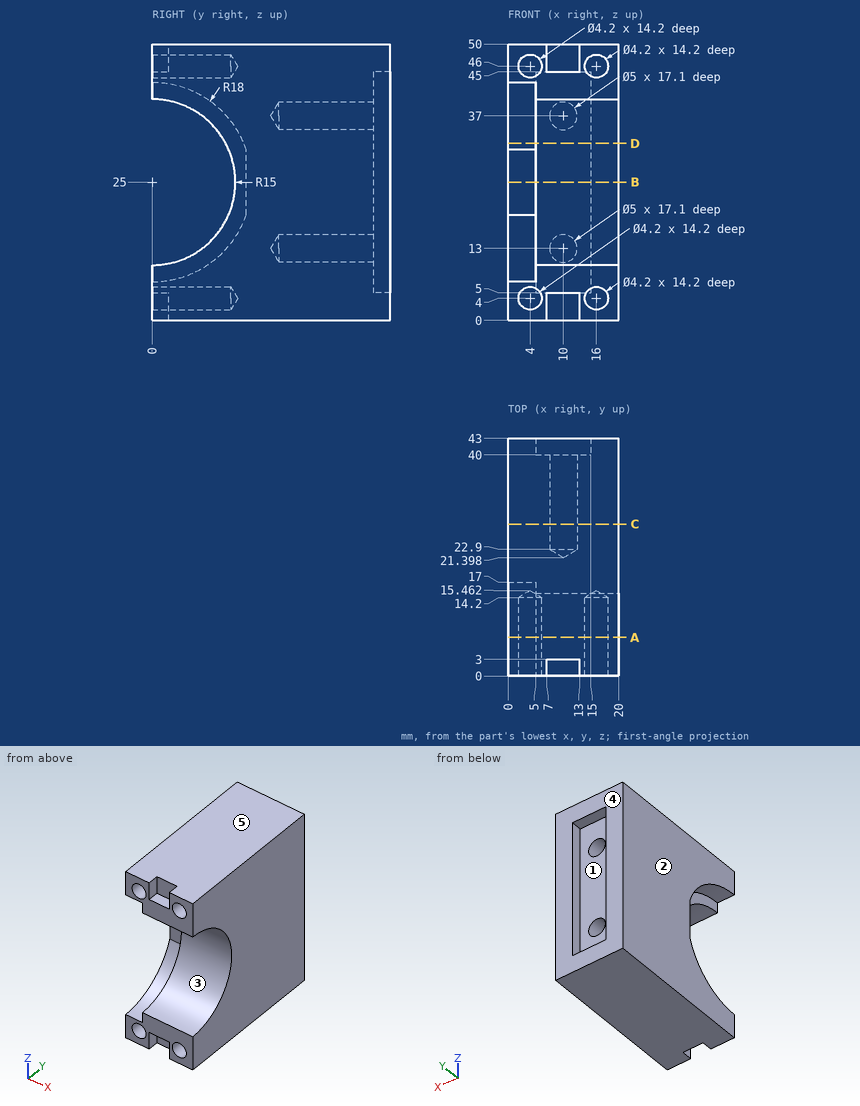
Study the drawing (mm; zero at the part's minimum x, y, z) and answer. A direction names the side the tool comes from. Coordinates: 2 decimals unless noted, no trailing zeros. Loops run counter-clockwise (first coordinate to the right, second up) from the corner with the lowest first, then second, coordinate; pieces in that order, holes last. Notation, with made-up numbers: (-22.5, -14.5) -> (26.5, -14.5) arc R32 ccw to (26.5, 14.5) -> close; hole circle Ø10 at (78, -14.75). An arc over 180 degrees is marked (long way). Answer as CSV lines item,"result".
1) For a pull along Z with two mould halves and no side action, classify the marked faces 3, 4 and 5 as released by +Z, released by -Z, zero draft, split by the parting line, or undercut.
A:
face 3,"undercut"
face 4,"zero draft"
face 5,"released by +Z"
2) The part is cut by section B-B (z = 25). Give the vertices of the cut face in (x, y), and give its area (3 significant figures).
A:
outline,"(0, 17) -> (5, 17) -> (5, 15) -> (20, 15) -> (20, 43) -> (15, 43) -> (15, 40) -> (5, 40) -> (5, 43) -> (0, 43) -> close"
area,"520 mm²"
3) The part is cut by section D-D (z = 32). Give the vertices of the cut face in (x, y).
A:
outline,"(0, 16.58) -> (5, 16.58) -> (5, 13.27) -> (20, 13.27) -> (20, 43) -> (15, 43) -> (15, 40) -> (5, 40) -> (5, 43) -> (0, 43) -> close"
4) The part is cut by section A-A (y = 7). Give the vertices of the cut face in (x, z), and give its area (3 significant figures).
A:
outline,"(0, 0) -> (20, 0) -> (20, 11.73) -> (5, 11.73) -> (5, 8.42) -> (0, 8.42) -> close; (0, 41.58) -> (5, 41.58) -> (5, 38.27) -> (20, 38.27) -> (20, 50) -> (0, 50) -> close; hole circle Ø4.2 at (4, 4); hole circle Ø4.2 at (4, 46); hole circle Ø4.2 at (16, 4); hole circle Ø4.2 at (16, 46)"
area,"381 mm²"
5) The part is cut by section C-C (y = 27.5). Give the vertices of the cut face in (x, z).
A:
outline,"(0, 0) -> (20, 0) -> (20, 50) -> (0, 50) -> close; hole circle Ø5 at (10, 13); hole circle Ø5 at (10, 37)"
6) For the marked faces 1 and 2, determine the directions among +Z, -Z, +X, -X, +Y, -Y from which every point of the face is accessible in a straight line to the end or side of a thin tool.
A:
face 1,"+Y"
face 2,"+Z, -Z, -X, +Y, -Y"
7) Flat-ended cylindrical pins translate along their axes: pin 1 (2.5 mm diameter, centred on x = 11.5, y = 1, fed in from -Z); pin 2 (13.5 mm diameter, centred on y = 7.5, z = 27.5, fed in from -X); pin 3 (1.5 mm diameter, centred on x = 1.5, z = 23, fed in from -Y); pin 4 (4 mm diameter, centred on x = 16, z = 46, fed in from -Y). Find the tip coordinate at first contact, or state that the pin passes through.
A:
pin 1,"stops at z = 5"
pin 2,"passes through"
pin 3,"stops at y = 17"
pin 4,"stops at y = 14.26"
8) Straight lines are drawn through the part: probe 1 along X at (y, z) = (10, 46); probe 2 along Z at (x, y) = (10, 27.75); probe 3 along X at (y, z) = (30, 37). For each, find the intervals that lie inside material, in ascending order.
A:
probe 1,"x = 0 to 1.9, 6.1 to 13.9, 18.1 to 20"
probe 2,"z = 0 to 10.5, 15.5 to 34.5, 39.5 to 50"
probe 3,"x = 0 to 7.5, 12.5 to 20"
